```python
from build123d import *

# Parameters (mm, degrees)
SKETCH1_W           = 150
SKETCH1_H           = 150
SKETCH1_W_2         = 140
SKETCH1_H_2         = 140
BOSS_EXTRUDE1_DEPTH = 608
FILLET1_R           = 10
FILLET2_R           = 5
SKETCH2_R           = 18
CUT_EXTRUDE1_DEPTH  = 644.944096953
SKETCH3_W           = 86
SKETCH3_H           = 55
CUT_EXTRUDE2_DEPTH  = 10
FILLET3_R           = 10


with BuildPart() as part:
    # Sketch1 → Boss-Extrude1 (new body)
    with BuildSketch(Plane.XY):
        with Locations((75, 75)):
            Rectangle(SKETCH1_W, SKETCH1_H)
        with Locations((75, 75)):
            Rectangle(SKETCH1_W_2, SKETCH1_H_2, mode=Mode.SUBTRACT)
    extrude(amount=BOSS_EXTRUDE1_DEPTH)

    # Fillet1
    fillet1_edges = [part.edges().sort_by_distance(p)[0] for p in [
        (0, 150, 304),
        (150, 150, 304),
        (150, 0, 304),
        (0, 0, 304),
    ]]
    fillet(fillet1_edges, radius=FILLET1_R)

    # Fillet2
    fillet2_edges = [part.edges().sort_by_distance(p)[0] for p in [
        (5, 145, 304),
        (5, 5, 304),
        (145, 5, 304),
        (145, 145, 304),
    ]]
    fillet(fillet2_edges, radius=FILLET2_R)

    # Sketch2 → Cut-Extrude1 (cut, through all)
    with BuildSketch(Plane.ZY):
        with Locations((574, 75)):
            Circle(SKETCH2_R)
    extrude(amount=-CUT_EXTRUDE1_DEPTH, mode=Mode.SUBTRACT)

    # Sketch3 → Cut-Extrude2 (cut)
    with BuildSketch(Plane.XZ):
        with Locations((75, 580.5)):
            Rectangle(SKETCH3_W, SKETCH3_H)
    extrude(amount=-CUT_EXTRUDE2_DEPTH, mode=Mode.SUBTRACT)

    # Fillet3
    fillet3_edges = [part.edges().sort_by_distance(p)[0] for p in [
        (32, 2.5, 553),
        (118, 2.5, 553),
    ]]
    fillet(fillet3_edges, radius=FILLET3_R)


solid = part.part
```
Geometry check sheet. Reference: the model listing, model coordinates, mm. A direction names the side the tool comes from. Round coordinates to 2 decimals unless told otherwise and drop trailing zeros. Write each loop counter-clockwise with the first axis right and the second up, starting at its lowest first coordinate (ties: lowest second). Pieces come first, ordered by that corner, then holes. Notation, with made-up numbers: (81.5, 17) - (89.5, 17) arc R22 ccw to (89.5, 33) - close; hole circle Ø2 at (65.25, 13). An arc over 180 degrees is marked (long way). Write each question's results on one line, items separated by ' | '.
(1) Draft check along X on faces 1 (the face through (146.99, 2.85, 308.26)), 2 (the face through (74, 0, 300)), 3 (the face through (35.01, 2.54, 555.85)). Enter one of: pulls with the +X half, pulls with the -X half, needs draft (parallel to the pull), parting line crosses it, or undercut.
Computed:
face 1: pulls with the +X half | face 2: needs draft | face 3: undercut
(2) Thickness scan on probe 1 along X at (y, z) = (102.5, 401); probe 2 along X at (y, z) = (141, 507). Record the ranges inside material, lowest first. Write a range as from..to.
Computed:
probe 1: x = 0..5, 145..150 | probe 2: x = 0.05..5.1, 144.9..149.95
(3) Sectioned sample at A-A, the plane x = 95. Enter the section's corners in (y, z).
Computed:
outline: (0, 0) - (5, 0) - (5, 553) - (0, 553) - close; (145, 0) - (150, 0) - (150, 608) - (145, 608) - close
(4) Set-up check for faces 4 (the face through (150, 74, 300)), 5 (the face through (74, 145, 300)), 6 (the face through (115.15, 2.54, 556.01)): record each of +Z, -Z, +X, -X, +Y, -Y from which the full face is reachable in a straight line by a thin tool's end or side.
Computed:
face 4: +Z, -Z, +X, +Y, -Y | face 5: +Z, -Z | face 6: +Z, -Y
(5) Sectioned sample at C-C, the plane y = 75. Enter the section's corners in (x, z), plus the area to 3 significant figures.
Computed:
outline: (0, 0) - (5, 0) - (5, 556) - (0, 556) - close; (0, 592) - (5, 592) - (5, 608) - (0, 608) - close; (145, 0) - (150, 0) - (150, 556) - (145, 556) - close; (145, 592) - (150, 592) - (150, 608) - (145, 608) - close | area: 5,720 mm^2
(6) Depth check by flat-ended pin: pin 1 Ø5.5 at (x, y) = (83, 3) entering from +Z; pin 2 Ø5.5 at (y, z) = (3, 591.5) entering from -X; pin 3 Ø1.5 at (y, z) = (3, 586) entering from +X. Enter the tip coordinate at first touch or a pass-through.
Computed:
pin 1: stops at z = 553 | pin 2: stops at x = 0.95 | pin 3: stops at x = 147.81
(7) Sectioned sample at D-D, the plane z = 185. Enter the section's corners in (x, y), plus the area to 3 significant figures.
Computed:
outline: (0, 10) arc R10 ccw to (10, 0) - (140, 0) arc R10 ccw to (150, 10) - (150, 140) arc R10 ccw to (140, 150) - (10, 150) arc R10 ccw to (0, 140) - close; hole (5, 10) arc R5 ccw to (10, 5) - (140, 5) arc R5 ccw to (145, 10) - (145, 140) arc R5 ccw to (140, 145) - (10, 145) arc R5 ccw to (5, 140) - close | area: 2,840 mm^2
(8) Sectioned sample at B-B, the plane z = 574. Enter the section's corners in (x, y).
Computed:
outline: (0, 10) arc R10 ccw to (10, 0) - (32, 0) - (32, 5) - (10, 5) arc R5 cw to (5, 10) - (5, 57) - (0, 57) - close; (0, 93) - (5, 93) - (5, 140) arc R5 cw to (10, 145) - (140, 145) arc R5 cw to (145, 140) - (145, 93) - (150, 93) - (150, 140) arc R10 ccw to (140, 150) - (10, 150) arc R10 ccw to (0, 140) - close; (118, 0) - (140, 0) arc R10 ccw to (150, 10) - (150, 57) - (145, 57) - (145, 10) arc R5 cw to (140, 5) - (118, 5) - close
